```python
from build123d import *

# Parameters (mm, degrees)
SKETCH1_W           = 1020
SKETCH1_H           = 480
BOSS_EXTRUDE1_DEPTH = 108
SHELL1_T            = -10
SKETCH2_R           = 18.75
CUT_EXTRUDE1_DEPTH  = 10


with BuildPart() as part:
    # Sketch1 → Boss-Extrude1 (new body)
    with BuildSketch(Plane.XY):
        Rectangle(SKETCH1_W, SKETCH1_H)
    extrude(amount=BOSS_EXTRUDE1_DEPTH)

    # Shell1
    shell1_openings = [part.faces().sort_by_distance(p)[0] for p in [
        (-510, 0, 54),
        (510, 0, 54),
    ]]
    offset(amount=SHELL1_T, openings=shell1_openings, kind=Kind.INTERSECTION)

    # Sketch2 → Cut-Extrude1 (cut)
    with BuildSketch(Plane(origin=(0, 0, 0), x_dir=(-1, 0, 0), z_dir=(0, 0, -1))):
        with Locations((-397.470896816, 192.1875)):
            Circle(SKETCH2_R)
        with Locations((-395.533103518, -192.1875)):
            Circle(SKETCH2_R)
        with Locations((465.091896482, -191.83711567)):
            Circle(SKETCH2_R)
        with Locations((465.091896482, 191.83711567)):
            Circle(SKETCH2_R)
    extrude(amount=-CUT_EXTRUDE1_DEPTH, mode=Mode.SUBTRACT)


solid = part.part
```
Geometry: final body of the model. Coordinates: model frame, mm. A direction names the side the tool comes from. Round coordinates to 2 decimals unless told otherwise and drop trailing zeros. Order: outer loops, then holes, each group sorted by start corner. A loop starts at its lowest first (then second) coordinate and runs counter-clockwise, first axis right, second up. Notation, with made-up numbers: M -39,42 L -7,42 A13 cw -7,52 Z; hole C -26,82.5 d7. An arc over 180 degrees is marked long. One line per item, written item: value.
(1) Pull-direction query (X, two-part tool) for faces 1 (the flat face through (-7, -240, 53)), 2 (the flat face through (-510, -18.9, 9.7)), 3 (the cylindrical face through (386.88, -208.82, 4.93)); classes: pulls with the +X half, pulls with the -X half, needs draft (parallel to the pull), parting line crosses it, or undercut.
Result sheet:
face 1: needs draft
face 2: pulls with the -X half
face 3: undercut
(2) Cut plane C-C (z = 81.5). Return the cut outline in (x, y), and give its area (3 significant figures).
Result sheet:
outline: M -510,-240 L 510,-240 L 510,-230 L -510,-230 Z; M -510,230 L 510,230 L 510,240 L -510,240 Z
area: 20,400 mm2
(3) Cut plane A-A (y = -128.5). Return the cut outline in (x, z).
Result sheet:
outline: M -510,0 L 510,0 L 510,10 L -510,10 Z; M -510,98 L 510,98 L 510,108 L -510,108 Z
(4) Line query: probe 1 along Y at (x, z) = (-339.5, 51); probe 2 along Z at (x, y) = (-110, -33.5). Output: solid intervals per line, ascending. Write a range as [from, to].
Result sheet:
probe 1: [-240, -230], [230, 240]
probe 2: [0, 10], [98, 108]
(5) Cut plane B-B (x = 106). Return the cut outline in (y, z).
Result sheet:
outline: M -240,0 L 240,0 L 240,108 L -240,108 Z; hole M -230,10 L 230,10 L 230,98 L -230,98 Z
(6) Reachability of faces 4 (the flat face through (510, -18.9, 9.7)), 5 (the flat face through (-7, 3, 10)), 6 (the cylindrical face through (412.35, 180.78, 4.93)) from +Z, -Z, +X, -X, +Y, -Y: full face, straight path, thin tool, end or side. Return the list, or none.
Result sheet:
face 4: +Z, -Z, +X, +Y, -Y
face 5: +X, -X
face 6: -Z
